```python
from build123d import *

# Parameters (mm, degrees)
SKETCH_1_W                   = 25
SKETCH_1_H                   = 60
EXTRUDE_1_DEPTH              = 6
CHAMFER_1_SIZE               = 2
HOLE_WIZARD_M5_1_D           = 5.5
HOLE_WIZARD_M5_1_DEPTH       = 12.4
HOLE_WIZARD_M5_1_CBORE_D     = 10
HOLE_WIZARD_M5_1_CBORE_DEPTH = 5.7
HOLE_WIZARD_M5_1_TIP         = 1.652366702
HOLE_WIZARD_M5_2_D           = 5.5
HOLE_WIZARD_M5_2_DEPTH       = 12.4
HOLE_WIZARD_M5_2_CBORE_D     = 10
HOLE_WIZARD_M5_2_CBORE_DEPTH = 5.7
HOLE_WIZARD_M5_2_TIP         = 1.652366702


with BuildPart() as part:
    # 草图1 → 凸台-拉伸1 (new, symmetric)
    with BuildSketch(Plane.XY):
        Rectangle(SKETCH_1_W, SKETCH_1_H)
    extrude(amount=EXTRUDE_1_DEPTH, both=True)

    # 倒角1
    chamfer_1_edges = [part.edges().sort_by_distance(p)[0] for p in [
        (12.5, -30, 0),
        (-12.5, -30, 0),
        (-12.5, 30, 0),
        (12.5, 30, 0),
    ]]
    chamfer(chamfer_1_edges, length=CHAMFER_1_SIZE)

    # M5 六角圆柱头螺钉的柱形沉头孔1
    with Locations(Plane(origin=(0, 0, -6), x_dir=(-1, 0, 0), z_dir=(0, 0, -1))):
        with Locations((6.5, 20), (6.5, -20)):
            CounterBoreHole(HOLE_WIZARD_M5_1_D / 2, HOLE_WIZARD_M5_1_CBORE_D / 2, HOLE_WIZARD_M5_1_CBORE_DEPTH, depth=HOLE_WIZARD_M5_1_DEPTH)
            with Locations((0, 0, -(HOLE_WIZARD_M5_1_DEPTH + HOLE_WIZARD_M5_1_TIP / 2))):  # 118° drill point
                Cone(0, HOLE_WIZARD_M5_1_D / 2, HOLE_WIZARD_M5_1_TIP, mode=Mode.SUBTRACT)

    # M5 六角圆柱头螺钉的柱形沉头孔2
    with Locations(Plane.XY.offset(6)):
        with Locations((6.5, 20), (6.5, -20)):
            CounterBoreHole(HOLE_WIZARD_M5_2_D / 2, HOLE_WIZARD_M5_2_CBORE_D / 2, HOLE_WIZARD_M5_2_CBORE_DEPTH, depth=HOLE_WIZARD_M5_2_DEPTH)
            with Locations((0, 0, -(HOLE_WIZARD_M5_2_DEPTH + HOLE_WIZARD_M5_2_TIP / 2))):  # 118° drill point
                Cone(0, HOLE_WIZARD_M5_2_D / 2, HOLE_WIZARD_M5_2_TIP, mode=Mode.SUBTRACT)


solid = part.part
```
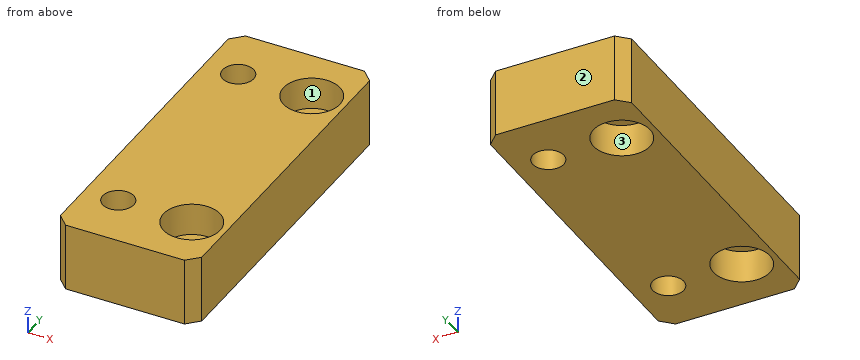
Input: part model. Units: mm. Frame: model coordinates. Face numbers are marked on the shaded views. A direction names the side the tool comes from. Coordinates: 2 decimals unless noted, no trailing zeros. Write each loop counter-clockwise with the first axis right and the second up, starting at its lowest first coordinate (ties: lowest second). Pieces come first, ordered by that corner, then holes. Notation, with made-up numbers: (72, 48.25) - (118, 48.25) arc R28 ccw to (118, 66.25) - close; hole circle Ø11 at (-28.5, 55). An arc over 180 degrees is marked (long way). Put each result on its own line as item: value. Start each with the question number.
1) Contact query for flat-ended pins moving along their axis: pin 1 (5 mm diameter, centred on x = 6.5, y = 20, fed in from -Z); pin 2 (8 mm diameter, centred on x = -6.5, y = 20, fed in from -Z); pin 3 (7 mm diameter, centred on x = 6.5, y = -20, fed in from +Z). Output: stop coordinate, or through.
2) Ray query, L1, parallel to Y at x = 6.5, z = -3.75; L2, parallel to Y at x = -6.5, z = -3; L3, parallel to X at y = 22.5, z = -3.5. Return the intervals inside material, ascending.
3) Cut plane C-C (x = -6.5). Return the cut outline in (y, z).
4) Cut plane A-A (z = 3.75). Return the cut outline in (x, y), plus the area to 3 significant figures.
5) Cut plane B-B (y = 20). Return the cut outline in (x, z), plus the area to 3 significant figures.
6) Reachability of the marked faces 1, 2 and 3 from +Z, -Z, +X, -X, +Y, -Y: full face, straight path, thin tool, end or side. Return the list, or none.
Resolved:
1. pin 1: passes through
1. pin 2: stops at z = -0.3
1. pin 3: stops at z = 0.3
2. L1: y = -30 to -22.75, -17.25 to 17.25, 22.75 to 30
2. L2: y = -30 to -25, -15 to 15, 25 to 30
2. L3: x = -12.5 to -10.83, -2.17 to 5.35, 7.65 to 12.5
3. outline: (-30, -6) - (-25, -6) - (-25, -0.3) - (-22.75, -0.3) - (-22.75, 6) - (-30, 6) - close; (-17.25, -0.3) - (-15, -0.3) - (-15, -6) - (15, -6) - (15, -0.3) - (17.25, -0.3) - (17.25, 6) - (-17.25, 6) - close; (22.75, -0.3) - (25, -0.3) - (25, -6) - (30, -6) - (30, 6) - (22.75, 6) - close
4. outline: (-12.5, -28) - (-10.5, -30) - (10.5, -30) - (12.5, -28) - (12.5, 28) - (10.5, 30) - (-10.5, 30) - (-12.5, 28) - close; hole circle Ø5.5 at (-6.5, -20); hole circle Ø5.5 at (-6.5, 20); hole circle Ø10 at (6.5, -20); hole circle Ø10 at (6.5, 20)
4. area: 1,290 mm2
5. outline: (-12.5, -6) - (-11.5, -6) - (-11.5, -0.3) - (-9.25, -0.3) - (-9.25, 6) - (-12.5, 6) - close; (-3.75, -0.3) - (-1.5, -0.3) - (-1.5, -6) - (3.75, -6) - (3.75, 0.3) - (1.5, 0.3) - (1.5, 6) - (-3.75, 6) - close; (9.25, -6) - (12.5, -6) - (12.5, 6) - (11.5, 6) - (11.5, 0.3) - (9.25, 0.3) - close
5. area: 117 mm2
6. face 1: +Z
6. face 2: +Z, -Z, +X, -X, +Y
6. face 3: -Z
